Source: CAD feature listing. Evaluate the final solid. Frame: model axes, mm. A direction names the side the tool comes from. Coordinates: 2 decimals unless noted, no trailing zeros. Loops run counter-clockwise (first coordinate to the right, second up) from the corner with the lowest first, then second, coordinate; pieces in that order, holes last.
Item 1: Section query C-C, the plane z = 7. Return the cut outline in (x, y).
Item 2: Pin query (flat end, axial travel): pin 1 Ø1 at (y, z) = (-20, 25.5) entering from +X; pin 2 Ø5 at (x, y) = (0.5, -23) entering from +Z; pin 3 Ø5.5 at (y, z) = (-22.5, 66.5) entering from +X. Return the tip coordinate at first contact, or that it passes through.
Item 3: Section query A-A, the plane y = 0. Return the cut outline in (x, z).
Item 4: Reachability of faces 1 (the flat face through (0, -25, 65)), 2 (the flat face through (-25, 5, 68)), 3 (the flat face through (-36.33, 26.464, 4.93)) from +Z, -Z, +X, -X, +Y, -Y: full face, straight path, thin tool, end or side. Return the list, or none.
Item 5: Line query: probe 1 along X at (y, z) = (-8, 9.5); probe 2 along Z at (x, y) = (-53, -13); probe 3 along Y at (x, z) = (-5, 13). Output: solid intervals per line, ascending.
Item 6: Section query B-B, the plane x = 0. Return the cut outline in (y, z), then the cut area to 3 significant figures.
Item 7: Section query D-D, the plane x = -49. Return the cut outline in (y, z).
Item 8: Pull-direction query (Y, two-part tool) for faces 4 (the cylindrical face through (-0.15, 35.05, 4.93)), 5 (the flat face through (1, -23, 0)), 6 (the cylindrical face through (-69.988, 0.55, 5.07)); classes: +Y half, -Y half, draft (parallel to the pull), parting line (faces both ways), or undercut.
```python
from build123d import *

# Parameters (mm, degrees)
FLANGE_PLATE_DEPTH      = 10
CYLINDER_BOSS_SKETCH_R  = 30
CYLINDER_BOSS_DEPTH     = 60
BORE_SKETCH_R           = 20
THROUGH_BORE_DEPTH      = 70
END_SLOTS_SKETCH_W      = 10
END_SLOTS_SKETCH_H      = 12.639410213
END_SLOTS_SKETCH_H_2    = 13.280913302
END_SLOTS_SKETCH_W_2    = 15.451741121
END_SLOTS_SKETCH_H_3    = 10
END_SLOTS_SKETCH_W_3    = 12.65016047
END_SLOTS_4X_DEPTH      = 5
MOUNTING_HOLES_SKETCH_R = 12.5
MOUNTING_HOLES_2X_DEPTH = 10


with BuildPart() as part:
    # Flange Plate Sketch → Flange Plate (new body)
    with BuildSketch(Plane.XY):
        with BuildLine():
            Line((9.143774129, 33.837267894), (62.730690194, 19.356587648))
            ThreePointArc((62.730690194, 19.356587648), (77.550875425, 0), (62.730690194, -19.356587648))
            Line((62.730690194, -19.356587648), (9.143774129, -33.837267894))
            ThreePointArc((9.143774129, -33.837267894), (-0.016117163, -35.050949261), (-9.174888429, -33.828844588))
            Line((-9.174888429, -33.828844588), (-62.735128416, -19.302506721))
            ThreePointArc((-62.735128416, -19.302506721), (-77.49983338, 0), (-62.735128416, 19.302506721))
            Line((-62.735128416, 19.302506721), (-9.174888429, 33.828844588))
            ThreePointArc((-9.174888429, 33.828844588), (-0.016117163, 35.050949261), (9.143774129, 33.837267894))
        make_face()
    extrude(amount=FLANGE_PLATE_DEPTH)

    # Cylinder Boss Sketch → Cylinder Boss (add)
    with BuildSketch(Plane.XY.offset(10)):
        Circle(CYLINDER_BOSS_SKETCH_R)
    extrude(amount=CYLINDER_BOSS_DEPTH)

    # Bore Sketch → Through Bore (cut)
    with BuildSketch(Plane.XY.offset(70)):
        Circle(BORE_SKETCH_R)
    extrude(amount=-THROUGH_BORE_DEPTH, mode=Mode.SUBTRACT)

    # End Slots Sketch → End Slots 4x (cut)
    with BuildSketch(Plane.XY.offset(70)):
        with Locations((0, 23.680294894)):
            Rectangle(END_SLOTS_SKETCH_W, END_SLOTS_SKETCH_H)
        with Locations((0, -23.359543349)):
            Rectangle(END_SLOTS_SKETCH_W, END_SLOTS_SKETCH_H_2)
        with Locations((-22.27412944, 0)):
            Rectangle(END_SLOTS_SKETCH_W_2, END_SLOTS_SKETCH_H_3)
        with Locations((23.674919765, 0)):
            Rectangle(END_SLOTS_SKETCH_W_3, END_SLOTS_SKETCH_H_3)
    extrude(amount=-END_SLOTS_4X_DEPTH, mode=Mode.SUBTRACT)

    # Mounting Holes Sketch → Mounting Holes 2x (cut)
    with BuildSketch(Plane.XY.offset(10)):
        with Locations((-57.5, 0)):
            Circle(MOUNTING_HOLES_SKETCH_R)
        with Locations((57.5, 0)):
            Circle(MOUNTING_HOLES_SKETCH_R)
    extrude(amount=-MOUNTING_HOLES_2X_DEPTH, mode=Mode.SUBTRACT)


solid = part.part
```
Verdict:
1. outline: (-62.74, -19.3) - (-9.17, -33.83) arc R35.05 ccw to (9.14, -33.84) - (62.73, -19.36) arc R20.05 ccw to (62.73, 19.36) - (9.14, 33.84) arc R35.05 ccw to (-9.17, 33.83) - (-62.74, 19.3) arc R20 ccw to start; hole circle Ø25 at (-57.5, 0); hole circle Ø40 at (0, 0); hole circle Ø25 at (57.5, 0)
2. pin 1: stops at x = 22.8
2. pin 2: stops at z = 65
2. pin 3: stops at x = 22.58
3. outline: (-77.5, 0) - (-70, 0) - (-70, 10) - (-77.5, 10) - close; (-45, 0) - (-20, 0) - (-20, 65) - (-30, 65) - (-30, 10) - (-45, 10) - close; (20, 0) - (45, 0) - (45, 10) - (30, 10) - (30, 65) - (20, 65) - close; (70, 0) - (77.55, 0) - (77.55, 10) - (70, 10) - close
4. face 1: +Z, +Y, -Y
4. face 2: +Z, +X, -X
4. face 3: +Z, -Z, -X, +Y
5. probe 1: x = -75.83 to -67.1, -47.9 to -18.33, 18.33 to 47.9, 67.1 to 75.89
5. probe 2: z = 0 to 10
5. probe 3: y = -29.58 to -19.36, 19.36 to 29.58
6. outline: (-35.05, 0) - (-20, 0) - (-20, 65) - (-30, 65) - (-30, 10) - (-35.05, 10) - close; (20, 0) - (35.05, 0) - (35.05, 10) - (30, 10) - (30, 65) - (20, 65) - close
6. area: 1,400 mm2
7. outline: (-23.03, 0) - (-9.17, 0) - (-9.17, 10) - (-23.03, 10) - close; (9.17, 0) - (23.03, 0) - (23.03, 10) - (9.17, 10) - close
8. face 4: +Y half
8. face 5: draft
8. face 6: undercut
